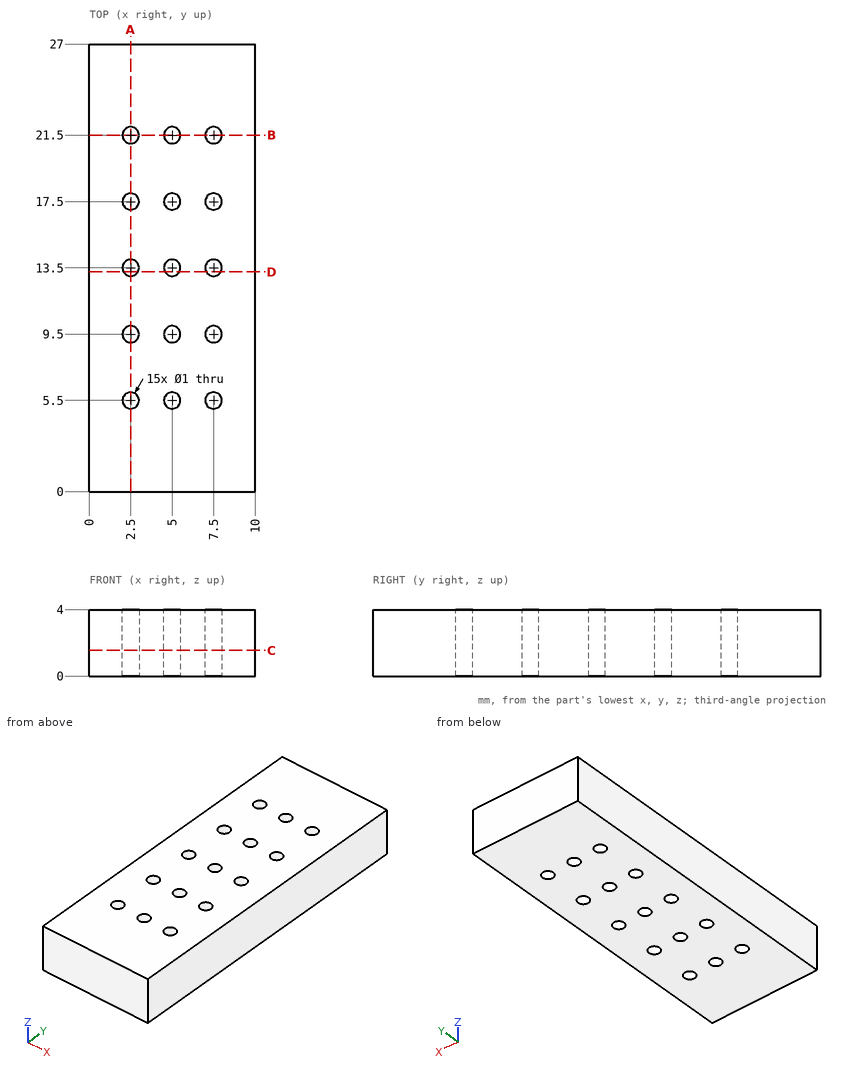
The drawing under review shows one solid part. Ordinate dimensions are in mm from its lowest x, y, z. Coordinates: 2 decimals unless noted, no trailing zeros. Order: outer loops, then holes, each group sorted by start corner. A loop starts at its lowest first (then second) coordinate and runs counter-clockwise, first axis right, second up. Notation, with made-up numbers: (-13.5, 56.5) -> (20.5, 56.5) arc R17 cw to (20.5, 74.5) -> close; hole circle Ø1 at (-32.75, 29.25). An arc over 180 degrees is marked (long way). Return JSON: item names as keys, results as strings.
1. For line 1 (X direction, y = 17.5, z = 1.7); line 2 (Y direction, x = 7.5, z = 1.3); line 3 (X direction, y = 5.75, z = 2.45), list the stretches that pass through material, from the lowest coordinate up. Write a range as from..to.
Answer block:
{"line 1": "0..2, 3..4.5, 5.5..7, 8..10", "line 2": "0..5, 6..9, 10..13, 14..17, 18..21, 22..27", "line 3": "0..2.07, 2.93..4.57, 5.43..7.07, 7.93..10"}
2. We need section A-A on x = 2.5. Write out the cut boundary in (y, z).
Answer block:
{"outline": "(0, 0) -> (5, 0) -> (5, 4) -> (0, 4) -> close; (6, 0) -> (9, 0) -> (9, 4) -> (6, 4) -> close; (10, 0) -> (13, 0) -> (13, 4) -> (10, 4) -> close; (14, 0) -> (17, 0) -> (17, 4) -> (14, 4) -> close; (18, 0) -> (21, 0) -> (21, 4) -> (18, 4) -> close; (22, 0) -> (27, 0) -> (27, 4) -> (22, 4) -> close"}
3. We need section C-C on z = 1.55. State how many separate pieces and enclosed holes the cut face has, and give its area (3 significant figures).
Answer block:
{"separate pieces": "1", "enclosed holes": "15", "area": "258 mm²"}
4. We need section D-D on y = 13.25. Write out the cut boundary in (x, z).
Answer block:
{"outline": "(0, 0) -> (2.07, 0) -> (2.07, 4) -> (0, 4) -> close; (2.93, 0) -> (4.57, 0) -> (4.57, 4) -> (2.93, 4) -> close; (5.43, 0) -> (7.07, 0) -> (7.07, 4) -> (5.43, 4) -> close; (7.93, 0) -> (10, 0) -> (10, 4) -> (7.93, 4) -> close"}
5. We need section B-B on y = 21.5. Write out the cut boundary in (x, z), and give its area (3 significant figures).
Answer block:
{"outline": "(0, 0) -> (2, 0) -> (2, 4) -> (0, 4) -> close; (3, 0) -> (4.5, 0) -> (4.5, 4) -> (3, 4) -> close; (5.5, 0) -> (7, 0) -> (7, 4) -> (5.5, 4) -> close; (8, 0) -> (10, 0) -> (10, 4) -> (8, 4) -> close", "area": "28.0 mm²"}
